Verification items for the finished model (mm, model axes). Give positions to 0.01 mm unless a question says otherwise; leave off trailing zeros. Write each loop counter-clockwise with the first axis right and the second up, starting at its lowest first coordinate (ties: lowest second). Pieces come first, ordered by that corner, then holes. Notation, with made-up numbers: M 22.25,-17 L 35.25,-17 A16 ccw 35.25,4 Z; hole C 82,75 d6. An arc over 180 degrees is marked long. Answer as a JSON object with one key per item and string values.
```python
from build123d import *

# Parameters (mm, degrees)
SKETCH1_R           = 15
BOSS_EXTRUDE1_DEPTH = 30


with BuildPart() as part:
    # Sketch1 → Boss-Extrude1 (new body)
    with BuildSketch(Plane.XY):
        with BuildLine():
            Line((137442.792186055, -173144.918087479), (137353.659547419, -173274.56556186))
            Line((137353.659547419, -173274.56556186), (137353.659547419, -173281.943182873))
            Line((137353.659547419, -173281.943182873), (137543.659547419, -173281.943182873))
            Line((137543.659547419, -173281.943182873), (137543.659547419, -173215.524161381))
            ThreePointArc((137543.659547419, -173215.524161381), (137541.785217916, -173205.086409641), (137536.396436674, -173195.952910355))
            Line((137536.396436674, -173195.952910355), (137490.250333171, -173142.34270129))
            ThreePointArc((137490.250333171, -173142.34270129), (137465.887841454, -173131.958027607), (137442.792186055, -173144.918087479))
        make_face()
        with Locations((137498.03455904, -173241.943182873)):
            Circle(SKETCH1_R, mode=Mode.SUBTRACT)
        with Locations((137428.03455904, -173241.943182873)):
            Circle(SKETCH1_R, mode=Mode.SUBTRACT)
    extrude(amount=BOSS_EXTRUDE1_DEPTH)


solid = part.part
```
1) Section check A-A on x = 137492.5. Record the boundary of the cut face in (y, z).
Completed:
{"outline": "M -173281.94,0 L -173255.88,0 L -173255.88,30 L -173281.94,30 Z; M -173228,0 L -173144.96,0 L -173144.96,30 L -173228,30 Z"}
2) Section check B-B on z = 5. Record the boundary of the cut face in (x, y).
Completed:
{"outline": "M 137353.66,-173281.94 L 137543.66,-173281.94 L 137543.66,-173215.52 A30 ccw 137536.4,-173195.95 L 137490.25,-173142.34 A30 ccw 137442.79,-173144.92 L 137353.66,-173274.57 Z; hole C 137428.03,-173241.94 d30; hole C 137498.03,-173241.94 d30"}
3) Section check C-C on y = -173186. Record the boundary of the cut face in (x, z).
Completed:
{"outline": "M 137414.55,0 L 137527.83,0 L 137527.83,30 L 137414.55,30 Z"}
4) Go/stop test with flat-tipped pins: pin 1 (1 mm diameter, centred on y = -173188, z = 4.5, fed in from +X); pin 2 (18 mm diameter, centred on x = 137498.03, y = -173241.94, fed in from -Z); pin 3 (6 mm diameter, centred on x = 137432, z = 14.5, fed in from +Y); pin 4 (1.5 mm diameter, centred on x = 137418.5, z = 13.5, fed in from +Y). Record where each tip stops, or that it passes through.
Completed:
{"pin 1": "stops at x = 137529.98", "pin 2": "passes through", "pin 3": "stops at y = -173156.25", "pin 4": "stops at y = -173179.16"}
5) Thickness scan on L1, parallel to Y at x = 137511.5, z = 20.5; L2, parallel to Y at x = 137511, z = 18.25; L3, parallel to X at y = -173214, z = 20. Record the ranges inside material, lowest first.
Completed:
{"L1": "y = -173281.94 to -173248.55, -173235.33 to -173167.03", "L2": "y = -173281.94 to -173249.49, -173234.4 to -173166.45", "L3": "x = 137395.3 to 137543.62"}
6) Release check for a two-part mould opening along X. For faces 1 (the face through (137504.96, -173255.25, 14.79)), 2 (the face through (137541.84, -173205.23, 14.79)), 3 (the face through (137466.27, -173131.94, 14.79)), 4 (the face through (137434.96, -173255.25, 14.79)) record: pulls with the +X half, pulls with the -X half, needs draft (parallel to the pull), parting line crosses it, or undercut.
Completed:
{"face 1": "undercut", "face 2": "pulls with the +X half", "face 3": "parting line crosses it", "face 4": "undercut"}
7) Section check D-D on x = 137447. Record the boundary of the cut face in (y, z), and give its area (3 significant figures).
Completed:
{"outline": "M -173281.94,0 L -173140.02,0 L -173140.02,30 L -173281.94,30 Z", "area": "4,260 mm2"}
